from build123d import *

# Parameters (mm, degrees)
SKETCH1_W           = 22
SKETCH1_H           = 71
SKETCH1_R           = 5
BOSS_EXTRUDE1_DEPTH = 4.5


with BuildPart() as part:
    # Sketch1 → Boss-Extrude1 (new body)
    with BuildSketch(Plane(origin=(0, 0, 0), x_dir=(1, 0, 0), z_dir=(0, 1, 0))):
        with Locations((11, 35.5)):
            Rectangle(SKETCH1_W, SKETCH1_H)
        with Locations(Location((11, 60, 0), (0, 0, 270))):
            Circle(SKETCH1_R, mode=Mode.SUBTRACT)
    extrude(amount=BOSS_EXTRUDE1_DEPTH)


solid = part.part
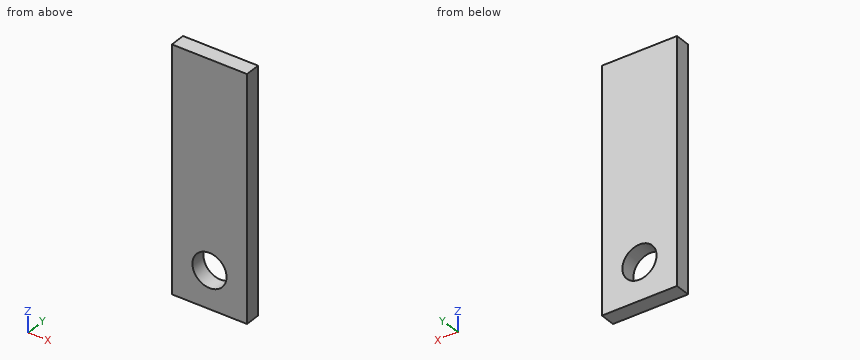
Check sheet for the modelled part. Datum: model origin and axes. Units: mm. Give positions to 0.01 mm unless a question says otherwise; leave off trailing zeros. Loops run counter-clockwise (first coordinate to the right, second up) from the corner with the lowest first, then second, coordinate; pieces in that order, holes last. Notation, with made-up numbers: M 13.5,-4.75 L 42.5,-4.75 A31 cw 42.5,23.25 Z; hole C 25,21.25 d10. An arc over 180 degrees is marked long. Answer as a JSON object with one key per item and string values. Group by question number.
Q1. Material ranges on line 1 along X through (y, z) = (1.25, -60); line 2 along Z through (x, y) = (12.25, 2); line 3 along Z through (x, y) = (15.5, 3.8), recorded low to high. Write a range as [from, to].
Q2. Go/stop test with a flat-tipped pin: P1, Ø6, axis at x = 11, z = -60, coming from the +Y side. Record where the tip stops, or that it passes through.
Q3. Cross-section at A-A on z = -60. Record the cut outline in (x, y), then the cut area to 3 significant figures.
Q4. Cross-section at C-C on y = 1.85. Record the cut outline in (x, z).
Q5. Cross-section at B-B on x = 11. Record the cut outline in (y, z).
Evaluation:
{
 "1": {"line 1": "x = [0, 6], [16, 22]", "line 2": "z = [-71, -64.84], [-55.16, 0]", "line 3": "z = [-71, -62.18], [-57.82, 0]"},
 "2": {"P1": "passes through"},
 "3": {"outline": "M 0,0 L 6,0 L 6,4.5 L 0,4.5 Z; M 16,0 L 22,0 L 22,4.5 L 16,4.5 Z", "area": "54.0 mm2"},
 "4": {"outline": "M 0,-71 L 22,-71 L 22,0 L 0,0 Z; hole C 11,-60 d10"},
 "5": {"outline": "M 0,-71 L 4.5,-71 L 4.5,-65 L 0,-65 Z; M 0,-55 L 4.5,-55 L 4.5,0 L 0,0 Z"}
}
